Input: part model. Units: mm. Frame: model coordinates. Give positions to 0.01 mm unless a question says otherwise; leave off trailing zeros. Order: outer loops, then holes, each group sorted by start corner. A loop starts at its lowest first (then second) coordinate and runs counter-clockwise, first axis right, second up. Notation, with made-up numbers: (-11.75, 27.25) - (9.25, 27.25) arc R23 cw to (9.25, 48.25) - close; hole circle Ø9 at (3.5, 7). An arc over 180 degrees is marked (long way). Answer in a Markdown table with one row per item. Add a question column.
1. Section query A-A on y = 18.5. Return loops of the section in (x, z), and give its area (3 significant figures).
2. Contact query for flat-ended pins moving along their axis: pin 1 (4 mm diameter, centred on y = 35, z = 10.5, fed in from -X); pin 2 (6 mm diameter, centred on y = -37.5, z = 21, fed in from +X); pin 3 (3 mm diameter, centred on y = 55.5, z = 57.5, fed in from +X). Output: stop coordinate, or through.
3. Section query B-B on z = 23. Return loops of the section in (x, y).
4. Ray query, line 1 (X direction, y = 1, z = 58); line 2 (X direction, y = -19, z = 40); line 3 (Y direction, x = -181.5, z = 28.5). Return the intervals inside material, ascending. Write a range as [from, to].
5. Section query C-C on x = 291.5. Return loops of the section in (y, z), and give its area (3 significant figures).
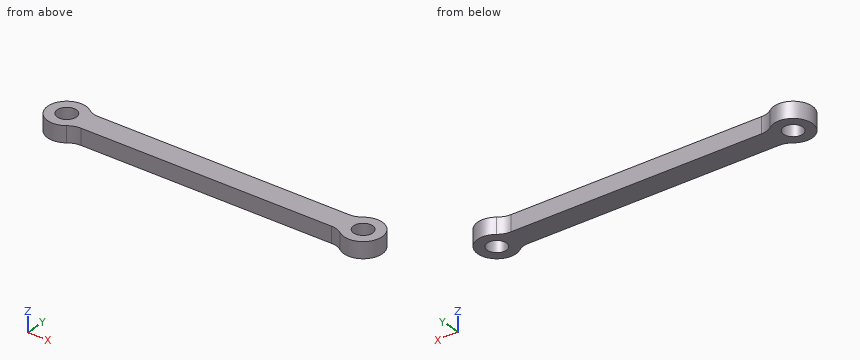
```python
from build123d import *

# Parameters (mm, degrees)
SKETCH1_R           = 50
BOSS_EXTRUDE1_DEPTH = 84


with BuildPart() as part:
    # Sketch1 → Boss-Extrude1 (new body)
    with BuildSketch(Plane.XY):
        with BuildLine():
            Line((-617.326495153, 59.809220037), (703.165599022, 59.809220037))
            ThreePointArc((703.165599022, 59.809220037), (734.86369832, 64.966031031), (763.292575479, 79.904610019))
            ThreePointArc((763.292575479, 79.904610019), (923.419551935, 0), (763.292575479, -79.904610019))
            ThreePointArc((763.292575479, -79.904610019), (734.86369832, -64.966031031), (703.165599022, -59.809220037))
            Line((703.165599022, -59.809220037), (-617.326495153, -59.809220037))
            ThreePointArc((-617.326495153, -59.809220037), (-649.02459445, -64.966031031), (-677.453471609, -79.904610019))
            ThreePointArc((-677.453471609, -79.904610019), (-837.580448065, 0), (-677.453471609, 79.904610019))
            ThreePointArc((-677.453471609, 79.904610019), (-649.02459445, 64.966031031), (-617.326495153, 59.809220037))
        make_face()
        with Locations(Location((-737.580448065, 0, 0), (0, 0, 180))):
            Circle(SKETCH1_R, mode=Mode.SUBTRACT)
        with Locations(Location((823.419551935, 0, 0), (0, 0, 180))):
            Circle(SKETCH1_R, mode=Mode.SUBTRACT)
    extrude(amount=BOSS_EXTRUDE1_DEPTH)


solid = part.part
```
Answer:
| question | item | result |
|---|---|---|
| 1 | outline | (-835.85, 0) - (-784.03, 0) - (-784.03, 84) - (-835.85, 84) - close; (-691.13, 0) - (776.97, 0) - (776.97, 84) - (-691.13, 84) - close; (869.87, 0) - (921.69, 0) - (921.69, 84) - (869.87, 84) - close |
| 1 | area | 132,000 mm² |
| 2 | pin 1 | stops at x = -831.98 |
| 2 | pin 2 | stops at x = 917.28 |
| 2 | pin 3 | stops at x = 907.59 |
| 3 | outline | (-677.45, -79.9) arc R100 cw to (-617.33, -59.81) - (703.17, -59.81) arc R100 cw to (763.29, -79.9) arc R100 ccw (long way) to (763.29, 79.9) arc R100 cw to (703.17, 59.81) - (-617.33, 59.81) arc R100 cw to (-677.45, 79.9) arc R100 ccw (long way) to start; hole circle Ø100 at (-737.58, 0); hole circle Ø100 at (823.42, 0) |
| 4 | line 1 | x = [-837.58, -787.57], [-687.59, 773.43], [873.41, 923.41] |
| 4 | line 2 | x = [-835.76, -783.83], [-691.33, 777.17], [869.67, 921.6] |
| 4 | line 3 | y = [-59.81, 59.81] |
| 5 | outline | (-59.81, 0) - (59.81, 0) - (59.81, 84) - (-59.81, 84) - close |
| 5 | area | 10,000 mm² |
